from build123d import *

# Parameters (mm, degrees)
CUT_EXTRUDE_1_DEPTH      = 49.47682334
CUT_EXTRUDE_1_DEPTH_BACK = 49.47682334


with BuildPart() as part:
    # 扫描2: sweep along a path in Sketch 203
    with BuildLine(Plane.XY) as sweep_2_path:
        Line((44.3, 1.85), (4.3, 1.85))
        ThreePointArc((4.3, 1.85), (3.421730256, 2.030913567), (2.686457501, 2.544198517))
        ThreePointArc((2.686457501, 2.544198517), (-3.7, 0), (2.686457501, -2.544198517))
        ThreePointArc((2.686457501, -2.544198517), (3.421730256, -2.030913567), (4.3, -1.85))
        Line((4.3, -1.85), (48.3, -1.85))
    # 草图2 → 扫描2 (sweep)
    with BuildSketch(Plane(origin=(44.3, 1.85, 0), x_dir=(0, 0, 1), z_dir=(-1, 0, 0))):
        with BuildLine():
            Line((-1.849972973, -1.84), (1.849972973, -1.84))
            ThreePointArc((1.849972973, -1.84), (0, 0), (-1.849972973, -1.84))
        make_face()
    sweep(path=sweep_2_path.line)

    # 草图3 → 切除-拉伸1 (cut, two sides: drawn at the far end of the back side and taken through both)
    with BuildSketch(Plane.XY.offset(-CUT_EXTRUDE_1_DEPTH_BACK)):
        Polygon((44.3, 0.92), (42.982464131, 1.85), (48.31, 1.85), (48.31, -1.85), (46.975462056, -1.85), (48.3, -0.93), (46.982464131, 0), (42.975462056, 0), align=None)
    extrude(amount=CUT_EXTRUDE_1_DEPTH + CUT_EXTRUDE_1_DEPTH_BACK, mode=Mode.SUBTRACT)


solid = part.part
Work out the finished part from the listing and answer in its coordinate system (mm). A direction names the side the tool comes from. Give positions to 0.01 mm unless a question says otherwise; leave off trailing zeros. Order: outer loops, then holes, each group sorted by start corner. A loop starts at its lowest first (then second) coordinate and runs counter-clockwise, first axis right, second up. Notation, with made-up numbers: (71, -32.75) -> (122, -32.75) arc R29 cw to (122, -0.75) -> close; hole circle Ø9 at (-11.75, 31). An arc over 180 degrees is marked (long way). Answer as a JSON object with one key per item and string values. Group by question number.
1. A tool of negligible diameter and unlimited length cuts with its end or side. For faces 1 (the cylindrical face through (24.02, 1.85, 0.04)), 2 (the cylindrical face through (26.61, -1.85, 0.04)), 3 (the flat face through (47.66, -0.48, -0.03)), from which of +Z, -Z, +X, -X, +Y, -Y can it reach the whole face along a straight path? Write none if from no direction.
2. Consider line 1 along Y through (x, z) = (0, 0.2); line 2 along X through (y, z) = (-0.75, 0.75) (3 decimals); line 3 along X through (y, z) = (1.25, -0.3). Determine where each line is inside the solid, lowest interval first. Write a range as [from, to].
3. The mould has two halves that part along Y. Classify faces 4 (the flat face through (43.797, 1.275, -0.022)), 5 (the cylindrical face through (2.67, -0.35, 0.03)), 6 (the flat face through (47.78, -1.29, -0.02)): released by +Y, released by -Y, zero draft, split by the parting line, or undercut.
4. A flat-ended cylindrical pin translates along its axis: pin 1 Ø3 at (x, y) = (41, -2) entering from -Z. Find the tip coordinate at first contact, or state that the pin passes through.
5. Section A-A on x = 22 is taken. Determine the outline of the cut face in (y, z).
Result sheet:
{
 "1": {"face 1": "+X, +Y", "face 2": "+X, -Y", "face 3": "+Z, -Z, +X, +Y"},
 "2": {"line 1": "y = [-3.69, -1.86], [1.86, 3.69]", "line 2": "x = [-3.461, -1.702], [1.962, 48.045]", "line 3": "x = [-3.46, -1.38], [1.38, 43.83]"},
 "3": {"face 4": "released by +Y", "face 5": "undercut", "face 6": "released by -Y"},
 "4": {"pin 1": "stops at z = -1.78"},
 "5": {"outline": "(-0.01, -1.85) -> (-0.01, 1.85) arc R1.85 ccw to start; (0.01, -1.85) arc R1.85 ccw to (0.01, 1.85) -> close"}
}
